from build123d import *

# Parameters (mm, degrees)
SKETCH_1_R          = 7
EXTRUDE_1_DEPTH     = 8
SKETCH_2_R          = 4.191
EXTRUDE_2_DEPTH     = 41.4
SKETCH_3_R          = 3
EXTRUDE_3_DEPTH     = 16
CUT_EXTRUDE_1_DEPTH = 5


with BuildPart() as part:
    # 草图1 → 凸台-拉伸1 (new body)
    with BuildSketch(Plane.XY):
        with Locations((-26.159273046, -76.997288483)):
            Circle(SKETCH_1_R)
    extrude(amount=EXTRUDE_1_DEPTH)

    # 草图2 → 凸台-拉伸2 (add)
    with BuildSketch(Plane(origin=(0, 0, 0), x_dir=(-1, 0, 0), z_dir=(0, 0, -1))):
        with Locations(Location((26.159273046, -76.997288483, 0), (0, 0, 180))):
            Circle(SKETCH_2_R)
    extrude(amount=EXTRUDE_2_DEPTH)

    # 草图3 → 凸台-拉伸3 (add)
    with BuildSketch(Plane(origin=(0, 0, -41.4), x_dir=(-1, 0, 0), z_dir=(0, 0, -1))):
        with Locations(Location((26.159273046, -76.997288483, 0), (0, 0, 180))):
            Circle(SKETCH_3_R)
    extrude(amount=EXTRUDE_3_DEPTH)

    # 草图4 → 切除-拉伸1 (cut)
    with BuildSketch(Plane.XY.offset(8)):
        Polygon((-24.356132828, -72.744992787), (-28.940299035, -73.309575399), (-30.743439252, -77.561871096), (-27.962413264, -81.249584179), (-23.378247058, -80.685001566), (-21.57510684, -76.43270587), align=None)
    extrude(amount=-CUT_EXTRUDE_1_DEPTH, mode=Mode.SUBTRACT)


solid = part.part
Geometry: final body of the model. Coordinates: model frame, mm. A direction names the side the tool comes from. Give positions to 0.01 mm unless a question says otherwise; leave off trailing zeros. Write each loop counter-clockwise with the first axis right and the second up, starting at its lowest first coordinate (ties: lowest second). Pieces come first, ordered by that corner, then holes. Notation, with made-up numbers: M -30,-8 L -17,-8 A18 cw -17,17 Z; hole C 49,18.5 d1. An arc over 180 degrees is marked long. Answer in a Markdown table with one row per item. Add a question column.
(1) Ray query, line 1 (Z direction, x = -20.75, y = -81.25); line 2 (Z direction, x = -26.25, y = -80.5); line 3 (Y direction, x = -26.5, z = -38). Return the intervals inside material, ascending.
(2) Reachability of faces 4 (the flat face through (-23, -80, 0)), 5 (the flat face through (-22.95, -74.61, 5.54)), 6 (the cylindrical face through (-31.71, -81.26, 3.94)) from +Z, -Z, +X, -X, +Y, -Y: full face, straight path, thin tool, end or side. Return the list, or none.
(3) Mould query, pull axis Y, two halves, no side actions, for faces 1 (the flat face through (-29.83, -75.41, 5.54)), 2 (the cylindrical face through (-28.37, -79.025, -49.288)), 3 (the flat face through (-26, -77, -57.4)). Classes: +Y half, -Y half, draft (parallel to the pull), parting line (faces both ways), or undercut.
(4) Section B-B on y = -75.75. Return loops of the section in (x, z), and give its area (3 significant figures).
(5) Section A-A on x = -25. Return loops of the section in (y, z), and give its area (3 significant figures).
(6) Section D-D on y = -82.75. Return loops of the section in (x, z), and give its area (3 significant figures).
(7) Section C-C on z = -32. Return loops of the section in (x, y), and give its area (3 significant figures).
(8) First-contact query: pin 1 (2 mm diameter, centred on x = -27, z = -20.5, fed in from -Y); pin 2 (1.5 mm diameter, centred on x = -25, y = -72.5, fed in from -Z); pin 3 (8 mm diameter, centred on y = -72.5, z = -20.5, fed in from -X). Flat tips, straight axial feed; report the tip coordinate or a pass-through.
Result set:
| question | item | result |
|---|---|---|
| 1 | line 1 | z = 0 to 8 |
| 1 | line 2 | z = -41.4 to 3 |
| 1 | line 3 | y = -81.17 to -72.82 |
| 2 | face 4 | -Z |
| 2 | face 5 | +Z |
| 2 | face 6 | +Z, -Z |
| 3 | face 1 | undercut |
| 3 | face 2 | parting line |
| 3 | face 3 | draft |
| 4 | outline | M -33.05,0 L -30.16,0 L -30.16,-41.4 L -28.89,-41.4 L -28.89,-57.4 L -23.43,-57.4 L -23.43,-41.4 L -22.16,-41.4 L -22.16,0 L -19.27,0 L -19.27,8 L -22.09,8 L -22.09,3 L -29.98,3 L -29.98,8 L -33.05,8 Z |
| 4 | area | 489 mm^2 |
| 5 | outline | M -83.9,0 L -81.02,0 L -81.02,-41.4 L -79.76,-41.4 L -79.76,-57.4 L -74.23,-57.4 L -74.23,-41.4 L -72.97,-41.4 L -72.97,0 L -70.09,0 L -70.09,8 L -72.82,8 L -72.82,3 L -80.88,3 L -80.88,8 L -83.9,8 Z |
| 5 | area | 492 mm^2 |
| 6 | outline | M -30.15,0 L -22.17,0 L -22.17,8 L -30.15,8 Z |
| 6 | area | 63.8 mm^2 |
| 7 | outline | C -26.16,-77 d8.38 |
| 7 | area | 55.2 mm^2 |
| 8 | pin 1 | stops at y = -81.19 |
| 8 | pin 2 | stops at z = -41.4 |
| 8 | pin 3 | stops at x = -30.32 |
